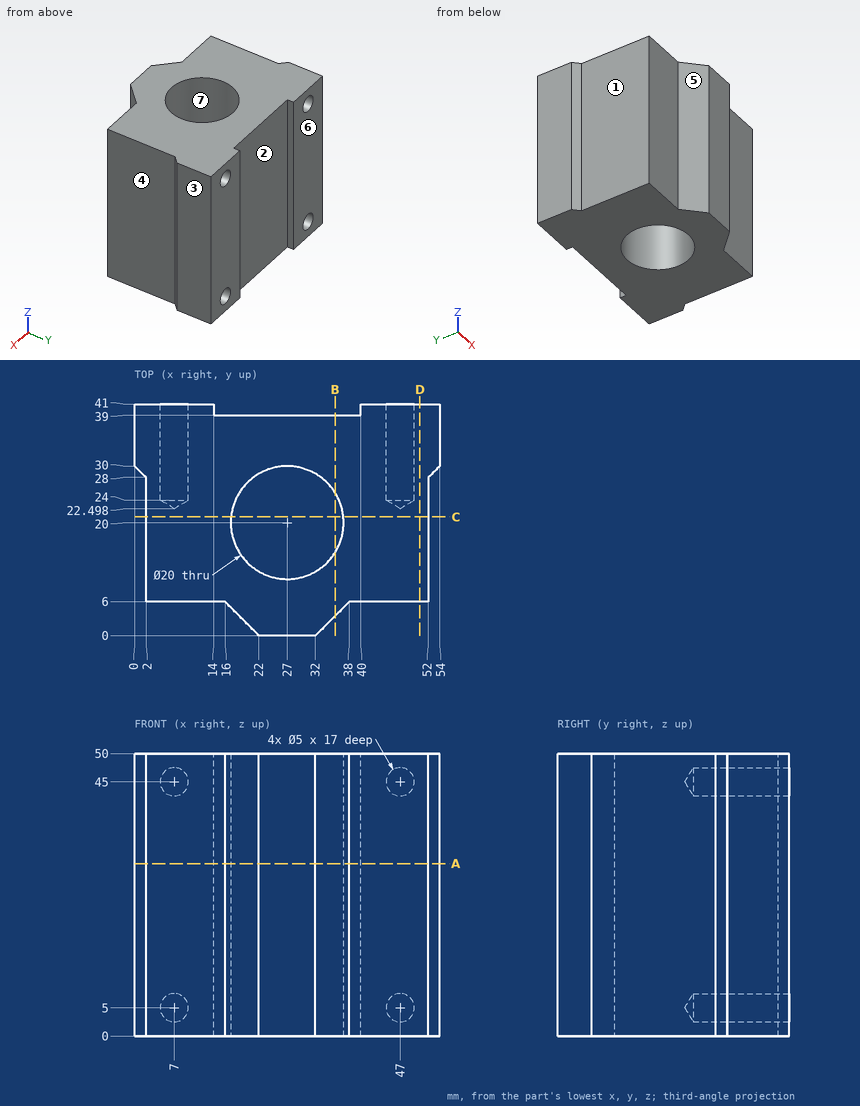
Design review of the part shown in the three views and the two pictorial views. Dimensions are in mm from the part's minimum x, y and z. A direction names the side the tool comes from. Give positions to 0.01 mm unless a question says otherwise; leave off trailing zeros. Loops run counter-clockwise (first coordinate to the right, second up) from the corner with the lowest first, then second, coordinate; pieces in that order, holes last. Notation, with made-up numbers: (18, -21.75) -> (70, -21.75) arc R25 cw to (70, 1.25) -> close; hole circle Ø3 at (60, 44). An arc over 180 degrees is marked (long way). Answer as a JSON object with one key per item and string values. Group by question number.
Q1. Draft analysis for pull direction Y (two halves, no side actions). For the marked faces 5, 6 and 7, state which applies: pulls with the +Y half, pulls with the -Y half, needs draft (parallel to the pull), parting line crosses it, or undercut.
Q2. Insertion check: pin 1 (4 mm diameter, centred on x = 46, z = 29, fed in from -Y); pin 2 (3 mm diameter, centred on y = 13.5, z = 9.5, fed in from +X); pin 3 (4 mm diameter, centred on x = 47, z = 5, fed in from +Y). Each pin has a flat end and moves straight along its axis. Give the tip position at first contact, or say it passes through.
Q3. Take a section at B-B (x = 35.5). Write out the cut boundary in (y, z).
Q4. Take a section at A-A (z = 30.5). Write out the cut boundary in (x, y).
Q5. Take a section at C-C (y = 21). Write out the cut boundary in (x, z), plus the area to 4 significant figures.
Q6. Wall thickness on line 1 along X through (y, z) = (36.25, 5); line 2 along Z through (x, y) = (7, 28.5); line 3 along Y through (x, z) = (27, 22): over which ranges is each line inside the solid? List them lowest first.
Q7. Tool access review of the marked faces 1, 2, 3 and 4: name each direction out of +Z, -Z, +X, -X, +Y, -Y from which nothing blocks a thin tool from reaching the whole face with its end or side.
Q8. Take a section at D-D (x = 50.5). Write out the cut boundary in (y, z).
Answer below:
{
 "1": {"face 5": "pulls with the -Y half", "face 6": "pulls with the +Y half", "face 7": "undercut"},
 "2": {"pin 1": "stops at y = 6", "pin 2": "stops at x = 52", "pin 3": "stops at y = 23.7"},
 "3": {"outline": "(3.5, 0) -> (14.73, 0) -> (14.73, 50) -> (3.5, 50) -> close; (25.27, 0) -> (39, 0) -> (39, 50) -> (25.27, 50) -> close"},
 "4": {"outline": "(0, 30) -> (2, 28) -> (2, 6) -> (16, 6) -> (22, 0) -> (32, 0) -> (38, 6) -> (52, 6) -> (52, 28) -> (54, 30) -> (54, 41) -> (40, 41) -> (40, 39) -> (14, 39) -> (14, 41) -> (0, 41) -> close; hole circle Ø20 at (27, 20)"},
 "5": {"outline": "(2, 0) -> (17.05, 0) -> (17.05, 50) -> (2, 50) -> close; (36.95, 0) -> (52, 0) -> (52, 50) -> (36.95, 50) -> close", "area": "1,505 mm2"},
 "6": {"line 1": "x = 0 to 4.5, 9.5 to 44.5, 49.5 to 54", "line 2": "z = 0 to 2.5, 7.5 to 42.5, 47.5 to 50", "line 3": "y = 0 to 10, 30 to 39"},
 "7": {"face 1": "+Z, -Z, -X, -Y", "face 2": "+Z, -Z, +Y", "face 3": "+Z, -Z, +X, +Y, -Y", "face 4": "+Z, -Z, +X, -Y"},
 "8": {"outline": "(6, 0) -> (41, 0) -> (41, 50) -> (6, 50) -> close"}
}
